from build123d import *

# Parameters (mm, degrees)
BOSS_EXTRUDE1_START = -5
SKETCH2_R           = 7
BOSS_EXTRUDE1_DEPTH = 5
BOSS_EXTRUDE2_START = 40
SKETCH3_R           = 16
SKETCH3_R_2         = 15
BOSS_EXTRUDE2_DEPTH = 40


with BuildPart() as part:
    # Sketch1 → Revolve1 (revolve)
    with BuildSketch(Plane.XY, mode=Mode.PRIVATE) as revolve1_sk:
        with BuildLine():
            Line((0, 0), (39, 0))
            Line((39, 0), (39, 127.168593742))
            ThreePointArc((39, 127.168593742), (37.973366174, 137.248742828), (34.935623776, 146.914947034))
            Line((34.935623776, 146.914947034), (15, 193.29086769))
            Line((15, 193.29086769), (15, 236))
            Line((15, 236), (7, 236))
            Line((7, 236), (7, 191.64423404))
            Line((7, 191.64423404), (31, 135.813420404))
            Line((31, 135.813420404), (31, 8))
            Line((31, 8), (0, 8))
            Line((0, 8), (0, 0))
        make_face()
    revolve(revolve1_sk.sketch.rotate(Axis((0, 0, 0), (0, 1, 0)), 90), axis=Axis((0, 0, 0), (0, 1, 0)))

    # Sketch2 → Boss-Extrude1 (add)
    with BuildSketch(Plane(origin=(0, 236, 0), x_dir=(1, 0, 0), z_dir=(0, 1, 0)).offset(BOSS_EXTRUDE1_START)):
        with Locations(Location((0, 0, 0), (0, 0, 90))):
            Circle(SKETCH2_R)
    extrude(amount=BOSS_EXTRUDE1_DEPTH)

    # Sketch3 → Boss-Extrude2 (add)
    with BuildSketch(Plane(origin=(0, 196, 0), x_dir=(1, 0, 0), z_dir=(0, 1, 0)).offset(BOSS_EXTRUDE2_START)):
        with Locations(Location((0, 0, 0), (0, 0, 270))):
            Circle(SKETCH3_R)
        with Locations(Location((0, 0, 0), (0, 0, 90))):
            Circle(SKETCH3_R_2, mode=Mode.SUBTRACT)
    extrude(amount=-BOSS_EXTRUDE2_DEPTH)


solid = part.part
Work out the finished part from the listing and answer in its coordinate system (mm). A direction names the side the tool comes from. Coordinates: 2 decimals unless noted, no trailing zeros. Loops run counter-clockwise (first coordinate to the right, second up) from the corner with the lowest first, then second, coordinate; pieces in that order, holes last. Notation, with made-up numbers: M -30,-10 L -18,-10 A13 ccw -18,12 Z; hole C -3.75,52 d2. An arc over 180 degrees is marked long. Answer in a Markdown table with one row per item. Add a question column.
1. A tool of negligible diameter and unlimited length cuts with its end or side. For faces 5 (the cylindrical face through (6.21, 211.05, -3.23)), 6 (the flat face through (-1, 0, -1)), from which of +Z, -Z, +X, -X, +Y, -Y can it reach the whole face along a straight path? Write none if from no direction.
2. Find section A-A, the plane y = 102.5. Write down the section's boundary in (x, z).
3. Consider L1, parallel to Y at x = 0, z = -3; L2, parallel to X at y = 205, z = 0; L3, parallel to X at y = 86, z = -1. Determine where each line is inside the solid, lowest interval first.
4. The mould has two halves that part along Y. Classify faces 1 (the flat face through (0, 231, 0)), 2 (the flat face through (0, 236, 0)), 3 (the flat face through (0, 8, 0)), 4 (the cylindrical face through (-15.62, 216.28, -3.47)): pulls with the +Y half, pulls with the -Y half, needs draft (parallel to the pull), parting line crosses it, or undercut.
5. Flat-ended cylindrical pins translate along their axes: P1, Ø7, axis at x = 0, z = 3.5, coming from the -Y side; P2, Ø8, axis at y = 75, z = -5, coming from the +X side; P3, Ø3, axis at x = 12, z = -23.5, coming from the +Y side; P4, Ø1, axis at x = 28.5, y = 70, coming from the -Z side. Find the tip coordinate at first contact, or state that the pin passes through.
Reported:
| question | item | result |
|---|---|---|
| 1 | face 5 | none |
| 1 | face 6 | +Z, -Z, +X, -X, -Y |
| 2 | outline | C 0,0 d78; hole C 0,0 d62 |
| 3 | L1 | y = 0 to 8, 231 to 236 |
| 3 | L2 | x = -16 to -7, 7 to 16 |
| 3 | L3 | x = -38.99 to -30.98, 30.98 to 38.99 |
| 4 | face 1 | undercut |
| 4 | face 2 | pulls with the +Y half |
| 4 | face 3 | undercut |
| 4 | face 4 | needs draft |
| 5 | P1 | stops at y = 0 |
| 5 | P2 | stops at x = 38.99 |
| 5 | P3 | stops at y = 170.29 |
| 5 | P4 | stops at z = -27.15 |
